from build123d import *

# Parameters (mm, degrees)
M10X1_0_TAPPED_HOLE1_D = 9
SKETCH4_R              = 3
CUT_EXTRUDE1_DEPTH     = 47.829477896


with BuildPart() as part:
    # Sketch1 → Revolve1 (revolve)
    with BuildSketch(Plane.XY, mode=Mode.PRIVATE) as revolve1_sk:
        Polygon((20, 0), (26, 0), (26, 19), (18, 19), (18, 29), (0, 29), (0, 17), (5, 17), (20, 11), align=None)
    revolve(revolve1_sk.sketch.rotate(Axis((0, 29.712230849, 0), (0, -1, 0)), 180), axis=Axis((0, 29.712230849, 0), (0, -1, 0)))

    # M10x1.0 Tapped Hole1 (through all)
    with Locations(Plane(origin=(0, 29, 0), x_dir=(1, 0, 0), z_dir=(0, 1, 0))):
        with Locations((0, 0)):
            Hole(M10X1_0_TAPPED_HOLE1_D / 2)

    # Sketch4 → Cut-Extrude1 (cut, through all)
    with BuildSketch(Plane(origin=(0, 0, 0), x_dir=(0, 0, -1), z_dir=(1, 0, 0))):
        with Locations(Location((0, 9, 0), (0, 0, 270.000000001))):
            Circle(SKETCH4_R)
    extrude(amount=-CUT_EXTRUDE1_DEPTH, mode=Mode.SUBTRACT)


solid = part.part
Work out the finished part from the listing and answer in its coordinate system (mm). A direction names the side the tool comes from. Give positions to 0.01 mm unless a question says otherwise; leave off trailing zeros. Loops run counter-clockwise (first coordinate to the right, second up) from the corner with the lowest first, then second, coordinate; pieces in that order, holes last. Notation, with made-up numbers: (72, -11) -> (90, -11) arc R25 ccw to (90, 2) -> close; hole circle Ø2 at (82, -35.5). An arc over 180 degrees is marked (long way). Use a Markdown table: item, result. Add a question column.
1) For a pull along Y with two mould halves and no side action, classify faces 1 (the flat face through (-5, 19, -18)), 2 (the flat face through (13.4, 0, 15.3)), 3 (the cylindrical face through (-23, 12, 0)) as +Y half, -Y half, draft (parallel to the pull), parting line (faces both ways), or undercut.
2) The part is cut by section D-D, the plane y = 10. Determine the outline of the cut face in (x, z), plus the area to 3 significant figures.
3) Consider line 1 along Z through (x, y) = (0, 4.5); line 2 along Z through (x, y) = (0, 25). Determine where each line is inside the solid, lowest interval first.
4) The part is cut by section A-A, the plane z = 0. Determine the outline of the cut face in (x, y).
5) The part is cut by section B-B, the plane x = 0. Determine the outline of the cut face in (y, z).
6) Each of these flat-tipped pins is pushed along its axis until it touches: P1, Ø5, axis at x = -1, z = 2, coming from the -Y side; P2, Ø6, axis at y = 10.5, z = 12.5, coming from the +X side; P3, Ø6, axis at x = -20.5, y = 16.5, coming from the +Z side. Where does it stop, or does it pass through?
7) The part is cut by section C-C, the plane x = -23. Determine the outline of the cut face in (y, z).
8) Which of the six approach directions +Z, -Z, +X, -X, +Y, -Y give full straight-line access (tool end or side, diameter ignored) to faces 4 (the cylindrical face through (13.267, 24.07, -12.165)), 5 (the cylindrical face through (19.98, 5.42, -0.88)), 6 (the cylindrical face through (20.633, 9.633, 15.821))?
Reported:
| question | item | result |
|---|---|---|
| 1 | face 1 | +Y half |
| 1 | face 2 | -Y half |
| 1 | face 3 | undercut |
| 2 | outline | (-25.85, -2.83) arc R26 ccw (long way) to (-25.85, 2.83) -> (-19.8, 2.83) arc R20 cw (long way) to (-19.8, -2.83) -> close |
| 2 | area | 833 mm^2 |
| 3 | line 1 | z = -26 to -20, 20 to 26 |
| 3 | line 2 | z = -18 to -4.5, 4.5 to 18 |
| 4 | outline | (-26, 0) -> (-20, 0) -> (-20, 6) -> (-26, 6) -> close; (-26, 12) -> (-17.5, 12) -> (-5, 17) -> (-4.5, 17) -> (-4.5, 29) -> (-18, 29) -> (-18, 19) -> (-26, 19) -> close; (4.5, 17) -> (5, 17) -> (20, 11) -> (20, 0) -> (26, 0) -> (26, 19) -> (18, 19) -> (18, 29) -> (4.5, 29) -> close |
| 5 | outline | (0, -26) -> (19, -26) -> (19, -18) -> (29, -18) -> (29, -4.5) -> (17, -4.5) -> (17, -5) -> (11, -20) -> (0, -20) -> close; (0, 20) -> (11, 20) -> (17, 5) -> (17, 4.5) -> (29, 4.5) -> (29, 18) -> (19, 18) -> (19, 26) -> (0, 26) -> close |
| 6 | P1 | stops at y = 17 |
| 6 | P2 | stops at x = 24.2 |
| 6 | P3 | stops at z = 19.23 |
| 7 | outline | (0, -12.12) -> (19, -12.12) -> (19, 12.12) -> (0, 12.12) -> close; hole circle Ø6 at (9, 0) |
| 8 | face 4 | +Y |
| 8 | face 5 | -Y |
| 8 | face 6 | +Y, -Y |
